The figure shows three views and two pictorial views of one solid part (mm, origin at its lowest corner). Answer the questions. Coordinates: 2 decimals unless noted, no trailing zeros. Loops run counter-clockwise (first coordinate to the right, second up) from the corner with the lowest first, then second, coordinate; pieces in that order, holes last. Notation, with made-up numbers: M 62.25,53.5 L 121.25,53.5 A28 cw 121.25,73.5 Z; hole C -26,19.25 d3. An arc over 180 degrees is marked long. Answer as a JSON object with one key per item and string values. Group by question number.
1. A cutting plane is placed at B-B on z = 6.5. Give the vertices of the cut face in (x, y), and give its area (3 significant figures).
2. A cutting plane is placed at A-A on y = 46. Give the vertices of the cut face in (x, z), and give its area (3 significant figures).
3. Given pin 1 (6 mm diameter, centred on y = 11, z = 2.5, fed in from -X); pin 2 (1 mm diameter, centred on x = 169, z = 6.5, fed in from +Y); pin 3 (1.5 mm diameter, centred on x = 145, z = 11, fed in from +Y), each flat-ended and moving along its own axis, determine where each tip first touches the part or whether it passes through.
4. Straight lines are drawn through the part: L1, parallel to X at y = 17.5, z = 8.25; L2, parallel to X at y = 12, z = 7.25; L3, parallel to Y at x = 74, z = 0.5. For each, find the intervals that lie inside material, in ascending order.
5. A cutting plane is placed at C-C on x = 104. Give the vertices of the cut face in (y, z).
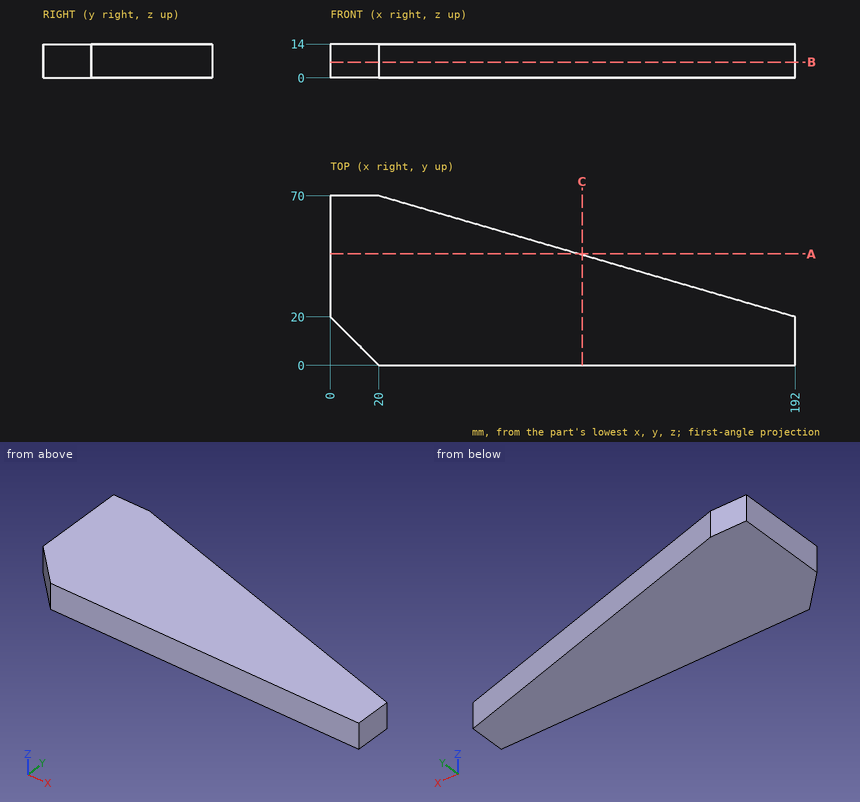
From the geometry:
{
 "1": {"outline": "M 0,20 L 20,0 L 192,0 L 192,20 L 20,70 L 0,70 Z", "area": "8,940 mm²"},
 "2": {"outline": "M 0,0 L 102.56,0 L 102.56,14 L 0,14 Z", "area": "1,440 mm²"},
 "3": {"pin 1": "stops at x = 6", "pin 2": "stops at y = 26.83", "pin 3": "stops at y = 33.88"},
 "4": {"L1": "x = 2.5 to 192", "L2": "x = 8 to 192", "L3": "y = 0 to 54.3"},
 "5": {"outline": "M 0,0 L 45.58,0 L 45.58,14 L 0,14 Z"}
}
